from build123d import *

# Parameters (mm, degrees)
SKETCH_1_W               = 75
SKETCH_1_H               = 75
EXTRUDE_1_DEPTH          = 1170
CUT_EXTRUDE_1_DEPTH      = 1170
CUT_EXTRUDE_2_DEPTH      = 2340
CUT_EXTRUDE_3_DEPTH      = 2341.600884388
CUT_EXTRUDE_3_DEPTH_BACK = 2341.600884388


with BuildPart() as part:
    # 草图1 → 凸台-拉伸1 (new, symmetric)
    with BuildSketch(Plane.XY):
        Rectangle(SKETCH_1_W, SKETCH_1_H)
    extrude(amount=EXTRUDE_1_DEPTH, both=True)

    # 草图2 → 切除-拉伸1 (cut, symmetric)
    with BuildSketch(Plane.XY):
        Polygon((-17.9, -36.8), (-16.55, -36.8), (-16.55, -34.5), (-25.45, -34.5), (-25.45, -36.8), (-24.1, -36.8), (-24.1, -37.5), (-17.9, -37.5), align=None)
        Polygon((16.55, -34.5), (16.55, -36.8), (17.9, -36.8), (17.9, -37.5), (24.1, -37.5), (24.1, -36.8), (25.45, -36.8), (25.45, -34.5), align=None)
    extrude(amount=CUT_EXTRUDE_1_DEPTH, both=True, mode=Mode.SUBTRACT)

    # 草图3 → 切除-拉伸2 (cut)
    with BuildSketch(Plane.XY.offset(1170)):
        Polygon((37.5, 2.6), (36.8, 2.6), (36.8, 4.45), (34.5, 4.45), (34.5, -4.45), (36.8, -4.45), (36.8, -2.6), (37.5, -2.6), align=None)
        Polygon((37.5, -17.9), (36.8, -17.9), (36.8, -16.55), (34.5, -16.55), (34.5, -25.45), (36.8, -25.45), (36.8, -24.1), (37.5, -24.1), align=None)
        Polygon((36.8, 24.1), (36.8, 25.45), (34.5, 25.45), (34.5, 16.55), (36.8, 16.55), (36.8, 17.9), (37.5, 17.9), (37.5, 24.1), align=None)
    cut_extrude_2 = extrude(amount=-CUT_EXTRUDE_2_DEPTH, mode=Mode.SUBTRACT)

    # 镜向1: 切除-拉伸2 across plane
    add(cut_extrude_2.mirror(Plane(origin=(0, 0, 0), x_dir=(0, 0, 1), z_dir=(1, 0, 0))), mode=Mode.SUBTRACT)

    # 草图4 → 切除-拉伸3 (cut, two sides: drawn at the far end of the back side and taken through both)
    with BuildSketch(Plane.XY.offset(1170).offset(-CUT_EXTRUDE_3_DEPTH_BACK)):
        Polygon((164.287302387, 109.214920955), (-15, 37.5), (-25, 33.5), (25, 33.5), (15, 37.5), (-164.287302387, 109.214920955), (-164.287302387, -276.981747517), (164.287302387, -276.981747517), align=None)
    extrude(amount=CUT_EXTRUDE_3_DEPTH + CUT_EXTRUDE_3_DEPTH_BACK, mode=Mode.SUBTRACT)


solid = part.part
Can you work these out from the model? Positions are in its coordinate system, mm. Give positions to 0.01 mm unless a question says otherwise; leave off trailing zeros. Order: outer loops, then holes, each group sorted by start corner. A loop starts at its lowest first (then second) coordinate and runs counter-clockwise, first axis right, second up. Notation, with made-up numbers: M -10,4.5 L 40,4.5 A10 cw 40,16.5 Z; hole C 16.5,45 d6. An arc over 180 degrees is marked long. Use a Markdown table: item, result. Add a question column.
Item 1: If I drill on L1, parallel to X at y = -17, z = 377.5; L2, parallel to Y at x = 23.5, z = 779; L3, parallel to Y at x = -7.5, z = -776, over which ranges is the centre line in solid material (lowest first)? Write a range as [from, to].
Item 2: Suppose I cut it at A-A (x = 3). List the corners of the cut face in (y, z) for me, then the cut area to 3 significant figures.
Item 3: We'd pull the mould along Y, two halves only. Please class faces 1 (the flat face through (0, -37.5, 16)), 2 (the flat face through (-1, 1, -1170)), 3 (the flat face through (0, 33.5, -16)): +Y half, -Y half, draft (parallel to the pull), parting line (faces both ways), or undercut.
Item 4: Will this pin go through, and if not, where does the flat tip stop? pin 1 (4 mm diameter, centred on x = 20.5, z = -746, fed in from -Y).
Answer sheet:
| question | item | result |
|---|---|---|
| 1 | L1 | x = [-37.5, -36.8], [-34.5, 34.5], [36.8, 37.5] |
| 1 | L2 | y = [-34.5, 33.5], [34.1, 37.5] |
| 1 | L3 | y = [-37.5, 33.5] |
| 2 | outline | M -37.5,-1170 L 33.5,-1170 L 33.5,1170 L -37.5,1170 Z |
| 2 | area | 166,000 mm² |
| 3 | face 1 | -Y half |
| 3 | face 2 | draft |
| 3 | face 3 | undercut |
| 4 | pin 1 | stops at y = -34.5 |
